Here's the drawing with two shaded views (mm, measured from the low corner). I have some questions. Give positions to 0.01 mm unless a question says otherwise; leave off trailing zeros. Write each loop counter-clockwise with the first axis right and the second up, starting at its lowest first coordinate (ties: lowest second). Pieces come first, ordered by that corner, then holes.
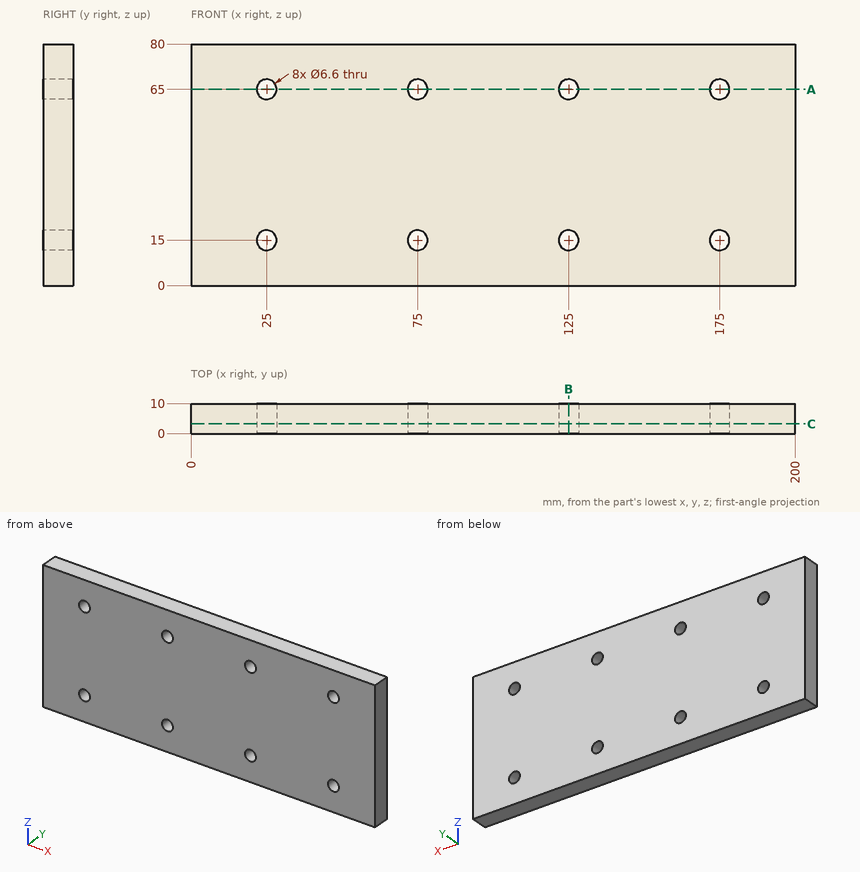
(1) Imagine slicing it at C-C, the plane y = 3.25. Give the number of separate pieces and of enclosed holes in the cut face, plus the area to 3 significant figures.
Returned:
separate pieces: 1
enclosed holes: 8
area: 15,700 mm2
(2) Will these pins go through, and if not, where does the flat tip stop? P1, Ø2, axis at y = 4.5, z = 72, coming from the -X side; P2, Ø4, axis at x = 175, z = 65, coming from the +Y side.
Returned:
P1: stops at x = 0
P2: passes through
(3) If I drill on L1, parallel to X at y = 6.25, z = 15; L2, parallel to Z at x = 175, y = 7; L3, parallel to X at y = 7.25, z = 62.5, over which ranges is the centre line in solid material (lowest first)?
Returned:
L1: x = 0 to 21.7, 28.3 to 71.7, 78.3 to 121.7, 128.3 to 171.7, 178.3 to 200
L2: z = 0 to 11.7, 18.3 to 61.7, 68.3 to 80
L3: x = 0 to 22.85, 27.15 to 72.85, 77.15 to 122.85, 127.15 to 172.85, 177.15 to 200
(4) Imagine slicing it at B-B, the plane x = 125. Write out the boundary of the cut face in (y, z).
Returned:
outline: (0, 0) - (10, 0) - (10, 11.7) - (0, 11.7) - close; (0, 18.3) - (10, 18.3) - (10, 61.7) - (0, 61.7) - close; (0, 68.3) - (10, 68.3) - (10, 80) - (0, 80) - close
(5) Imagine slicing it at A-A, the plane z = 65. Write out the boundary of the cut face in (x, y), plus the area to 3 significant figures.
Returned:
outline: (0, 0) - (21.7, 0) - (21.7, 10) - (0, 10) - close; (28.3, 0) - (71.7, 0) - (71.7, 10) - (28.3, 10) - close; (78.3, 0) - (121.7, 0) - (121.7, 10) - (78.3, 10) - close; (128.3, 0) - (171.7, 0) - (171.7, 10) - (128.3, 10) - close; (178.3, 0) - (200, 0) - (200, 10) - (178.3, 10) - close
area: 1,740 mm2
